Work out the finished part from the listing and answer in its coordinate system (mm). Face numbers are marked on the shaded views. A direction names the side the tool comes from. Coordinates: 2 decimals unless noted, no trailing zeros. Write each loop counter-clockwise with the first axis right and the second up, starting at its lowest first coordinate (ties: lowest second). Pieces come first, ordered by that corner, then holes. Notation, with made-up numbers: (-16.5, 20.25) - (31.5, 20.25) arc R13 ccw to (31.5, 42.25) - close; hole circle Ø5 at (48.5, 0.5). An arc over 180 degrees is marked (long way). Answer as a JSON object with one key per item and string values. Group by question number.
from build123d import *

# Parameters (mm, degrees)
ELBOW_PIPE_290_PROFILE_R          = 145
FLANGE_1_360X360X50_DEPTH         = 50
FLANGE_1_BOLT_HOLE_SKETCH_R       = 30
FLANGE_1_BOLT_HOLE_SKETCH_R_2     = 15
FLANGE_1_COUNTERBORES_4X_60_DEPTH = 10
SKETCH9_2_R                       = 15
FLANGE_1_BOLT_HOLES_4X_30_DEPTH   = 50
FLANGE_2_360X360X50_DEPTH         = 50
FLANGE_2_BOLT_HOLE_SKETCH_R       = 30
FLANGE_2_BOLT_HOLE_SKETCH_R_2     = 15
FLANGE_2_COUNTERBORES_4X_60_DEPTH = 10
SKETCH11_2_R                      = 15
FLANGE_2_BOLT_HOLES_4X_30_DEPTH   = 50
ELBOW_BORE_210_PROFILE_R          = 105
BORE_CHAMFER_10X45_SIZE           = 10


with BuildPart() as part:
    # Elbow Pipe _290: sweep along a path in Elbow Path Sketch
    with BuildLine(Plane.XY) as elbow_pipe_290_path:
        Line((0, 410), (0, 260))
        ThreePointArc((0, 260), (-76.152236891, 76.152236891), (-260, 0))
        Line((-260, 0), (-410, 0))
    # Elbow Pipe _290 profile (on start of the path) → Elbow Pipe _290 (sweep)
    with BuildSketch(Plane(origin=(0, 410, 0), x_dir=(0, 0, -1), z_dir=(0, -1, 0))):
        Circle(ELBOW_PIPE_290_PROFILE_R)
    sweep(path=elbow_pipe_290_path.line)

    # Flange 1 Sketch → Flange 1 360x360x50 (add)
    with BuildSketch(Plane(origin=(0, 410, 0), x_dir=(1, 0, 0), z_dir=(0, 1, 0))):
        with BuildLine():
            Line((-160, 180), (160, 180))
            ThreePointArc((160, 180), (174.142135624, 174.142135624), (180, 160))
            Line((180, 160), (180, -160))
            ThreePointArc((180, -160), (174.142135624, -174.142135624), (160, -180))
            Line((160, -180), (-160, -180))
            ThreePointArc((-160, -180), (-174.142135624, -174.142135624), (-180, -160))
            Line((-180, -160), (-180, 160))
            ThreePointArc((-180, 160), (-174.142135624, 174.142135624), (-160, 180))
        make_face()
    extrude(amount=-FLANGE_1_360X360X50_DEPTH)

    # Flange 1 Bolt Hole Sketch → Flange 1 Counterbores 4x_60 (cut)
    # profile 1 of 4: a face of its own
    with BuildSketch(Plane(origin=(0, 410, 0), x_dir=(1, 0, 0), z_dir=(0, 1, 0))):
        with Locations(Location((-130, 130, 0), (0, 0, 180))):
            Circle(FLANGE_1_BOLT_HOLE_SKETCH_R)
        with Locations(Location((-130, 130, 0), (0, 0, 180))):
            Circle(FLANGE_1_BOLT_HOLE_SKETCH_R_2, mode=Mode.SUBTRACT)
    # profile 2 of 4: a face of its own
    with BuildSketch(Plane(origin=(0, 410, 0), x_dir=(1, 0, 0), z_dir=(0, 1, 0))):
        with Locations(Location((-130, -130, 0), (0, 0, 180))):
            Circle(FLANGE_1_BOLT_HOLE_SKETCH_R)
        with Locations(Location((-130, -130, 0), (0, 0, 180))):
            Circle(FLANGE_1_BOLT_HOLE_SKETCH_R_2, mode=Mode.SUBTRACT)
    # profile 3 of 4: a face of its own
    with BuildSketch(Plane(origin=(0, 410, 0), x_dir=(1, 0, 0), z_dir=(0, 1, 0))):
        with Locations((130, -130)):
            Circle(FLANGE_1_BOLT_HOLE_SKETCH_R)
        with Locations((130, -130)):
            Circle(FLANGE_1_BOLT_HOLE_SKETCH_R_2, mode=Mode.SUBTRACT)
    # profile 4 of 4: a face of its own
    with BuildSketch(Plane(origin=(0, 410, 0), x_dir=(1, 0, 0), z_dir=(0, 1, 0))):
        with Locations((130, 130)):
            Circle(FLANGE_1_BOLT_HOLE_SKETCH_R)
        with Locations((130, 130)):
            Circle(FLANGE_1_BOLT_HOLE_SKETCH_R_2, mode=Mode.SUBTRACT)
    extrude(amount=-FLANGE_1_COUNTERBORES_4X_60_DEPTH, mode=Mode.SUBTRACT)

    # Sketch9_2 → Flange 1 Bolt Holes 4x_30 (cut)
    with BuildSketch(Plane(origin=(0, 410, 0), x_dir=(1, 0, 0), z_dir=(0, 1, 0))):
        with Locations(Location((-130, 130, 0), (0, 0, 180))):
            Circle(SKETCH9_2_R)
        with Locations(Location((130, 130, 0), (0, 0, 270))):
            Circle(SKETCH9_2_R)
        with Locations(Location((-130, -130, 0), (0, 0, 180))):
            Circle(SKETCH9_2_R)
        with Locations(Location((130, -130, 0), (0, 0, 270))):
            Circle(SKETCH9_2_R)
    extrude(amount=-FLANGE_1_BOLT_HOLES_4X_30_DEPTH, mode=Mode.SUBTRACT)

    # Flange 2 Sketch → Flange 2 360x360x50 (add)
    with BuildSketch(Plane.ZY.offset(410)):
        with BuildLine():
            Line((-160, 180), (160, 180))
            ThreePointArc((160, 180), (174.142135624, 174.142135624), (180, 160))
            Line((180, 160), (180, -160))
            ThreePointArc((180, -160), (174.142135624, -174.142135624), (160, -180))
            Line((160, -180), (-160, -180))
            ThreePointArc((-160, -180), (-174.142135624, -174.142135624), (-180, -160))
            Line((-180, -160), (-180, 160))
            ThreePointArc((-180, 160), (-174.142135624, 174.142135624), (-160, 180))
        make_face()
    extrude(amount=-FLANGE_2_360X360X50_DEPTH)

    # Flange 2 Bolt Hole Sketch → Flange 2 Counterbores 4x_60 (cut)
    # profile 1 of 4: a face of its own
    with BuildSketch(Plane.ZY.offset(410)):
        with Locations(Location((-130, 130, 0), (0, 0, 270))):
            Circle(FLANGE_2_BOLT_HOLE_SKETCH_R)
        with Locations(Location((-130, 130, 0), (0, 0, 270))):
            Circle(FLANGE_2_BOLT_HOLE_SKETCH_R_2, mode=Mode.SUBTRACT)
    # profile 2 of 4: a face of its own
    with BuildSketch(Plane.ZY.offset(410)):
        with Locations(Location((-130, -130, 0), (0, 0, 270))):
            Circle(FLANGE_2_BOLT_HOLE_SKETCH_R)
        with Locations(Location((-130, -130, 0), (0, 0, 270))):
            Circle(FLANGE_2_BOLT_HOLE_SKETCH_R_2, mode=Mode.SUBTRACT)
    # profile 3 of 4: a face of its own
    with BuildSketch(Plane.ZY.offset(410)):
        with Locations(Location((130, -130, 0), (0, 0, 90))):
            Circle(FLANGE_2_BOLT_HOLE_SKETCH_R)
        with Locations(Location((130, -130, 0), (0, 0, 90))):
            Circle(FLANGE_2_BOLT_HOLE_SKETCH_R_2, mode=Mode.SUBTRACT)
    # profile 4 of 4: a face of its own
    with BuildSketch(Plane.ZY.offset(410)):
        with Locations(Location((130, 130, 0), (0, 0, 90))):
            Circle(FLANGE_2_BOLT_HOLE_SKETCH_R)
        with Locations(Location((130, 130, 0), (0, 0, 90))):
            Circle(FLANGE_2_BOLT_HOLE_SKETCH_R_2, mode=Mode.SUBTRACT)
    extrude(amount=-FLANGE_2_COUNTERBORES_4X_60_DEPTH, mode=Mode.SUBTRACT)

    # Sketch11_2 → Flange 2 Bolt Holes 4x_30 (cut)
    with BuildSketch(Plane.ZY.offset(410)):
        with Locations(Location((130, 130, 0), (0, 0, 270))):
            Circle(SKETCH11_2_R)
        with Locations(Location((-130, 130, 0), (0, 0, 270))):
            Circle(SKETCH11_2_R)
        with Locations(Location((-130, -130, 0), (0, 0, 270))):
            Circle(SKETCH11_2_R)
        with Locations(Location((130, -130, 0), (0, 0, 90))):
            Circle(SKETCH11_2_R)
    extrude(amount=-FLANGE_2_BOLT_HOLES_4X_30_DEPTH, mode=Mode.SUBTRACT)

    # Elbow Bore _210: sweep along a path in Sketch1_2
    with BuildLine(Plane.XY) as elbow_bore_210_path:
        Line((0, 410), (0, 260))
        ThreePointArc((0, 260), (-76.152236891, 76.152236891), (-260, 0))
        Line((-260, 0), (-410, 0))
    # Elbow Bore _210 profile (on start of the path) → Elbow Bore _210 (sweep, cut)
    with BuildSketch(Plane(origin=(0, 410, 0), x_dir=(0, 0, -1), z_dir=(0, -1, 0))):
        Circle(ELBOW_BORE_210_PROFILE_R)
    sweep(path=elbow_bore_210_path.line, mode=Mode.SUBTRACT)

    # Bore Chamfer 10x45
    bore_chamfer_10x45_edges = [part.edges().sort_by_distance(p)[0] for p in [
        (-410, 0, 105),
        (0, 410, 105),
    ]]
    chamfer(bore_chamfer_10x45_edges, length=BORE_CHAMFER_10X45_SIZE)


solid = part.part
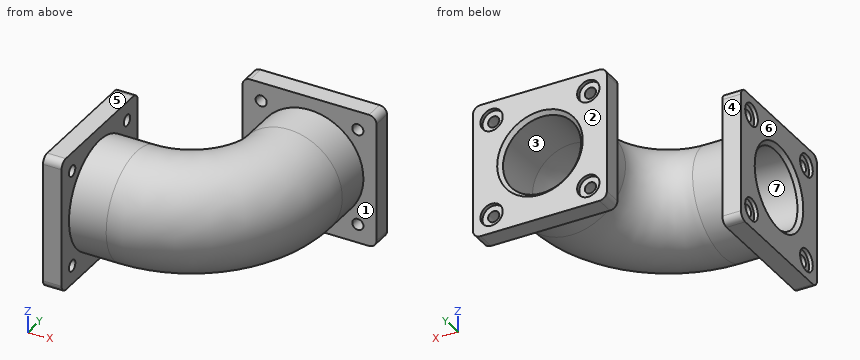
Q1. For a pull along Z with two mould halves and no side action, classify the marked faces 5, 6 and 7 as +Z half, -Z half, draft (parallel to the pull), parting line (faces both ways), or undercut.
Q2. Consider L1, parallel to Z at x = 130, y = 382.5; L2, parallel to Z at x = -130, y = 402.5; L3, parallel to Y at x = -291.5, z = 0. Determine where each line is inside the solid, lowest interval first. Write a range as from..to.
Q3. Flat-ended cylindrical pins translate along their axes: pin 1 Ø1.5 at (x, z) = (-331, 14) entering from -Y; pin 2 Ø3 at (x, y) = (-75, 235) entering from +Z; pin 3 Ø10 at (x, z) = (-264.5, 42) entering from -Y. Find the tip coordinate at first contact, or state that the pin passes through.
Q4. Section A-A on x = -130 is taken. Count the separate pieces of the cut face and the enclosed holes in it, plus the area to 3 significant figures.
Q5. A tool of negligible diameter and unlimited length cuts with its end or side. For the marked faces 1, 2, 3 and 4, from which of +Z, -Z, +X, -X, +Y, -Y can it reach the whole face along a straight path? Write none if from no direction.
Q6. Section C-C on x = -280.5 is taken. Determine the outline of the cut face in (y, z).
Numbers:
{
 "1": {"face 5": "+Z half", "face 6": "draft", "face 7": "undercut"},
 "2": {"L1": "z = -180..-145, -115..115, 145..180", "L2": "z = -180..-160, -100..100, 160..180", "L3": "y = -145..-105, 105..145"},
 "3": {"pin 1": "stops at y = -144.39", "pin 2": "stops at z = 125.96", "pin 3": "stops at y = -140.2"},
 "4": {"separate pieces": "3", "enclosed holes": "1", "area": "71,600 mm²"},
 "5": {"face 1": "none", "face 2": "+Z, -Z, +X, -X, +Y", "face 3": "+Y", "face 4": "+Z, -Z, -X, +Y"},
 "6": {"outline": "circle Ø290 at (0, 0); hole circle Ø210 at (0, 0)"}
}
